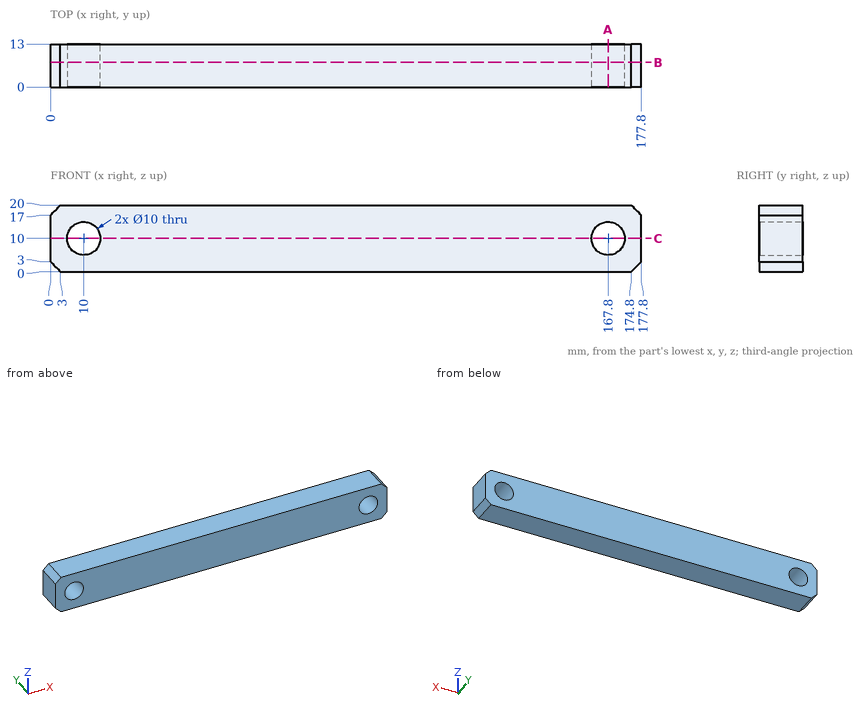
The figure shows three views and two pictorial views of one solid part (mm, origin at its lowest corner). Answer the questions. Round coordinates to 2 decimals unless told otherwise and drop trailing zeros. Order: outer loops, then holes, each group sorted by start corner. A loop starts at its lowest first (then second) coordinate and runs counter-clockwise, first axis right, second up. Notation, with made-up numbers: M -22,-4 L 21,-4 A15 ccw 21,12 Z; hole C 8,-21.5 d1. An arc over 180 degrees is marked long. Put each result on its own line as item: value. Start each with the question number.
Q1. Section A-A, the plane x = 167.8 is taken. Write down the section's boundary in (y, z).
Q2. Section C-C, the plane z = 10 is taken. Write down the section's boundary in (x, y).
Q3. Section B-B, the plane y = 7.5 is taken. Write down the section's boundary in (x, z).
Q4. Straight lines are drawn through the part: L1, parallel to X at y = 1.25, z = 5.75; L2, parallel to X at y = 8.75, z = 10.5; L3, parallel to Z at x = 167.8, y = 6.5. For each, find the intervals that lie inside material, in ascending order. Write a range as [from, to].
Findings below:
1. outline: M 0,0 L 13,0 L 13,5 L 0,5 Z; M 0,15 L 13,15 L 13,20 L 0,20 Z
2. outline: M 0,0 L 5,0 L 5,13 L 0,13 Z; M 15,0 L 162.8,0 L 162.8,13 L 15,13 Z; M 172.8,0 L 177.8,0 L 177.8,13 L 172.8,13 Z
3. outline: M 0,3 L 3,0 L 174.8,0 L 177.8,3 L 177.8,17 L 174.8,20 L 3,20 L 0,17 Z; hole C 10,10 d10; hole C 167.8,10 d10
4. L1: x = [0, 7.37], [12.63, 165.17], [170.43, 177.8]
4. L2: x = [0, 5.03], [14.97, 162.83], [172.77, 177.8]
4. L3: z = [0, 5], [15, 20]
